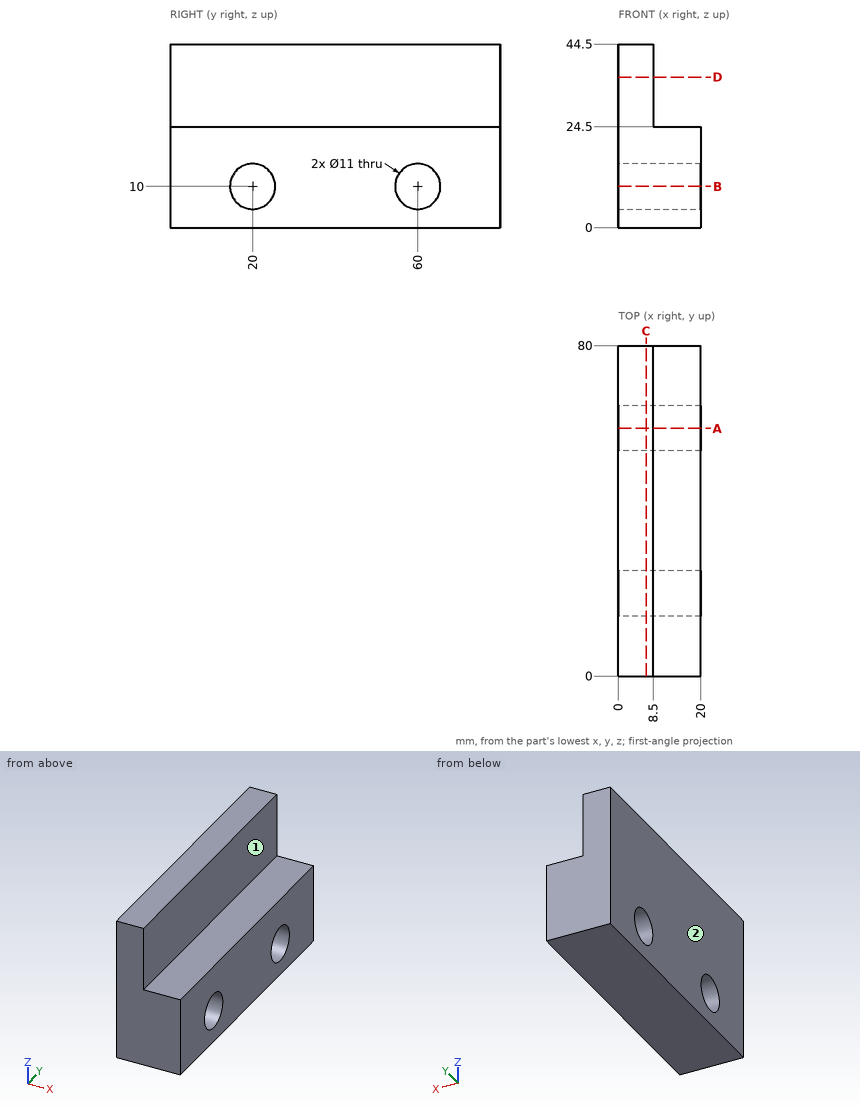
Study the drawing (mm; zero at the part's minimum x, y, z) and answer. A direction names the side the tool comes from. Round coordinates to 2 decimals unless told otherwise and drop trailing zeros. Write each loop counter-clockwise with the first axis right and the second up, starting at its lowest first coordinate (ties: lowest second). Pieces come first, ordered by that corner, then holes. Notation, with made-up numbers: (70, -35) - (89, -35) arc R12 cw to (89, -28) - close; hole circle Ø7 at (-28.5, 83.25). An arc over 180 degrees is marked (long way). Return JSON: item names as keys, results as strings. Group by question number.
Q1. Each of these flat-tipped pins is pushed along its axis until it touches: pin 1 Ø6 at (y, z) = (27.5, 37) entering from +X; pin 2 Ø9 at (x, y) = (16, 25) entering from +Z. Where does it stop, or does it pass through?
Q2. The part is cut by section A-A on y = 60. Write down the section's boundary in (x, z), then the cut area to 3 significant figures.
Q3. The part is cut by section D-D on z = 36.5. Write down the section's boundary in (x, y).
Q4. The part is cut by section B-B on z = 10. Write down the section's boundary in (x, y), then the cut area to 3 significant figures.
Q5. For the marked faces 1 and 2, determine the directions among +Z, -Z, +X, -X, +Y, -Y from which every point of the face is accessible in a straight line to the end or side of a thin tool.
Q6. Find the intervals of material crossed by L1, parallel to Y at x = 6, z = 10; L2, parallel to Z at x = 13, y = 47.5; L3, parallel to Y at x = 16.75, z = 6, in increasing order.
Q7. The part is cut by section C-C on x = 6.75. Write down the section's boundary in (y, z), then the cut area to 3 significant figures.
Solved:
{
 "1": {"pin 1": "x = 8.5", "pin 2": "z = 24.5"},
 "2": {"outline": "(0, 0) - (20, 0) - (20, 4.5) - (0, 4.5) - close; (0, 15.5) - (20, 15.5) - (20, 24.5) - (8.5, 24.5) - (8.5, 44.5) - (0, 44.5) - close", "area": "440 mm²"},
 "3": {"outline": "(0, 0) - (8.5, 0) - (8.5, 80) - (0, 80) - close"},
 "4": {"outline": "(0, 0) - (20, 0) - (20, 14.5) - (0, 14.5) - close; (0, 25.5) - (20, 25.5) - (20, 54.5) - (0, 54.5) - close; (0, 65.5) - (20, 65.5) - (20, 80) - (0, 80) - close", "area": "1,160 mm²"},
 "5": {"face 1": "+Z, +X, +Y, -Y", "face 2": "+Z, -Z, -X, +Y, -Y"},
 "6": {"L1": "0 to 14.5, 25.5 to 54.5, 65.5 to 80", "L2": "0 to 24.5", "L3": "0 to 16.23, 23.77 to 56.23, 63.77 to 80"},
 "7": {"outline": "(0, 0) - (80, 0) - (80, 44.5) - (0, 44.5) - close; hole circle Ø11 at (20, 10); hole circle Ø11 at (60, 10)", "area": "3,370 mm²"}
}
